Check sheet for the modelled part. Datum: model origin and axes. Units: mm. Face numbers are marked on the shaded views. A direction names the side the tool comes from. Coordinates: 2 decimals unless noted, no trailing zeros. Loops run counter-clockwise (first coordinate to the right, second up) from the corner with the lowest first, then second, coordinate; pieces in that order, holes last.
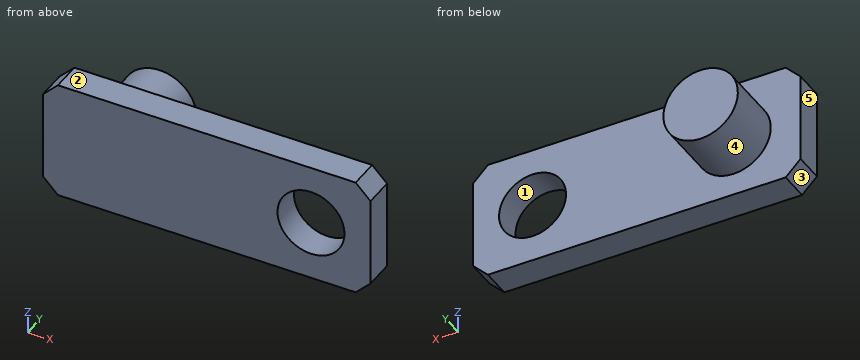
```python
from build123d import *

# Parameters (mm, degrees)
SKETCH1_W           = 22
SKETCH1_H           = 8
BOSS_EXTRUDE1_DEPTH = 2
SKETCH2_R           = 2.25
CUT_EXTRUDE1_DEPTH  = 12.874342087
SKETCH3_R           = 2.5
BOSS_EXTRUDE2_DEPTH = 4
CHAMFER1_SIZE       = 1


with BuildPart() as part:
    # Sketch1 → Boss-Extrude1 (new body)
    with BuildSketch(Plane(origin=(0, 0, 0), x_dir=(1, 0, 0), z_dir=(0, 1, 0))):
        Rectangle(SKETCH1_W, SKETCH1_H)
    extrude(amount=BOSS_EXTRUDE1_DEPTH)

    # Sketch2 → Cut-Extrude1 (cut, through all)
    with BuildSketch(Plane(origin=(0, 2, 0), x_dir=(1, 0, 0), z_dir=(0, 1, 0))):
        with Locations(Location((7, 0, 0), (0, 0, 270))):
            Circle(SKETCH2_R)
    extrude(amount=-CUT_EXTRUDE1_DEPTH, mode=Mode.SUBTRACT)

    # Sketch3 → Boss-Extrude2 (add)
    with BuildSketch(Plane(origin=(0, 2, 0), x_dir=(1, 0, 0), z_dir=(0, 1, 0))):
        with Locations(Location((-6.5, 0, 0), (0, 0, 90))):
            Circle(SKETCH3_R)
    extrude(amount=BOSS_EXTRUDE2_DEPTH)

    # Chamfer1
    chamfer1_edges = [part.edges().sort_by_distance(p)[0] for p in [
        (11, 1, 4),
        (-11, 1, 4),
        (-11, 1, -4),
        (11, 1, -4),
    ]]
    chamfer(chamfer1_edges, length=CHAMFER1_SIZE)


solid = part.part
```
1) Set-up check for the marked faces 4 and 5: record each of +Z, -Z, +X, -X, +Y, -Y from which the full face is reachable in a straight line by a thin tool's end or side.
Answer sheet:
face 4: +Y
face 5: +Z, -Z, -X, +Y, -Y
2) Scan lines: line 1 (Y direction, x = 0.5, z = -1.5); line 2 (X direction, y = 0.7, z = 0); line 3 (X direction, y = 0.65, z = 1.5). Record each from-to range of solid material in increasing order.
Answer sheet:
line 1: y = 0 to 2
line 2: x = -11 to 4.75, 9.25 to 11
line 3: x = -11 to 5.32, 8.68 to 11
3) Section check A-A on z = 0. Enter the section's corners in (x, y), plus the area to 3 significant figures.
Answer sheet:
outline: (-11, 0) - (4.75, 0) - (4.75, 2) - (-4, 2) - (-4, 6) - (-9, 6) - (-9, 2) - (-11, 2) - close; (9.25, 0) - (11, 0) - (11, 2) - (9.25, 2) - close
area: 55.0 mm2
4) Section check B-B on x = 7. Enter the section's corners in (y, z).
Answer sheet:
outline: (0, -4) - (2, -4) - (2, -2.25) - (0, -2.25) - close; (0, 2.25) - (2, 2.25) - (2, 4) - (0, 4) - close
5) Depth check by flat-ended pin: pin 1 (1.5 mm diameter, centred on y = 3.5, z = 0, fed in from -X); pin 2 (2.5 mm diameter, centred on x = 3, z = 0, fed in from +Y). Enter the tip coordinate at first touch or a pass-through.
Answer sheet:
pin 1: stops at x = -9
pin 2: stops at y = 2
6) Section check C-C on y = 1.4. Enter the section's corners in (x, z), plus the area to 3 significant figures.
Answer sheet:
outline: (-11, -3) - (-10, -4) - (10, -4) - (11, -3) - (11, 3) - (10, 4) - (-10, 4) - (-11, 3) - close; hole circle Ø4.5 at (7, 0)
area: 158 mm2
7) Mould release check, pull along Z, two halves, no side actions. Record for the marked faces 1, 2 and 3: +Z half, -Z half, draft (parallel to the pull), parting line (faces both ways), or undercut.
Answer sheet:
face 1: undercut
face 2: +Z half
face 3: -Z half
8) Section check D-D on x = -6.5. Enter the section's corners in (y, z).
Answer sheet:
outline: (0, -4) - (2, -4) - (2, -2.5) - (6, -2.5) - (6, 2.5) - (2, 2.5) - (2, 4) - (0, 4) - close
